Geometry: final body of the model. Coordinates: model frame, mm. A direction names the side the tool comes from. Coordinates: 2 decimals unless noted, no trailing zeros. Write each loop counter-clockwise with the first axis right and the second up, starting at its lowest first coordinate (ties: lowest second). Pieces come first, ordered by that corner, then holes.
from build123d import *

# Parameters (mm, degrees)
SKETCH1_W               = 1100
SKETCH1_H               = 500
SKETCH1_W_2             = 1000
SKETCH1_H_2             = 400
BOSS_EXTRUDE1_DEPTH     = 75
SKETCH2_W               = 50
SKETCH2_H               = 50
BOSS_EXTRUDE2_DEPTH     = 800
CUT_EXTRUDE1_DEPTH      = 1383.931668594
CUT_EXTRUDE1_DEPTH_BACK = 1383.931668594
SKETCH3_R               = 7.5


with BuildPart() as part:
    # Sketch1 → Boss-Extrude1 (new body)
    with BuildSketch(Plane(origin=(0, 0, 0), x_dir=(1, 0, 0), z_dir=(0, 1, 0))):
        Rectangle(SKETCH1_W, SKETCH1_H)
        Rectangle(SKETCH1_W_2, SKETCH1_H_2, mode=Mode.SUBTRACT)
    extrude(amount=BOSS_EXTRUDE1_DEPTH)

    # Sketch2 → Boss-Extrude2 (add)
    with BuildSketch(Plane.XZ):
        with Locations((-525, 225)):
            Rectangle(SKETCH2_W, SKETCH2_H)
        with Locations((525, 225)):
            Rectangle(SKETCH2_W, SKETCH2_H)
        with Locations((525, -225)):
            Rectangle(SKETCH2_W, SKETCH2_H)
        with Locations((-525, -225)):
            Rectangle(SKETCH2_W, SKETCH2_H)
    extrude(amount=BOSS_EXTRUDE2_DEPTH)

    # Sketch3 → Cut-Extrude1 (cut, two sides: drawn at the far end of the back side and taken through both)
    with BuildSketch(Plane.ZY.offset(550).offset(-CUT_EXTRUDE1_DEPTH_BACK)):
        with Locations(Location((0, 52.5, 0), (0, 0, 180))):
            Circle(SKETCH3_R)
    extrude(amount=CUT_EXTRUDE1_DEPTH + CUT_EXTRUDE1_DEPTH_BACK, mode=Mode.SUBTRACT)


solid = part.part
Item 1: Pin query (flat end, axial travel): pin 1 (15 mm diameter, centred on x = 525.5, z = -93, fed in from -Y). Return the tip coordinate at first contact, or that it passes through.
Derived:
pin 1: stops at y = 0
Item 2: Section A-A, the plane y = -232.5. Output: boundary loops of the cut face in (x, z), plus the area to 3 significant figures.
Derived:
outline: (-550, -250) - (-500, -250) - (-500, -200) - (-550, -200) - close; (-550, 200) - (-500, 200) - (-500, 250) - (-550, 250) - close; (500, -250) - (550, -250) - (550, -200) - (500, -200) - close; (500, 200) - (550, 200) - (550, 250) - (500, 250) - close
area: 10,000 mm2
Item 3: Section C-C, the plane x = -438. Output: boundary loops of the cut face in (y, z), plus the area to 3 significant figures.
Derived:
outline: (0, -250) - (75, -250) - (75, -200) - (0, -200) - close; (0, 200) - (75, 200) - (75, 250) - (0, 250) - close
area: 7,500 mm2
Item 4: Material intervals for probe 1 along Z at (x, y) = (516, 52); probe 2 along Y at (x, z) = (-532, 0); probe 3 along Z at (x, y) = (312, 21), sorted ascending.
Derived:
probe 1: z = -250 to -7.48, 7.48 to 250
probe 2: y = 0 to 45, 60 to 75
probe 3: z = -250 to -200, 200 to 250
Item 5: Pull-direction query (X, two-part tool) for faces 1 (the flat face through (-500, -394, -225)), 2 (the flat face through (550, -300, 205)), 3 (the flat face through (-550, -263, -205)), 4 (the flat face through (525, -394, -200)); classes: released by +X, released by -X, zero draft, split by the parting line, or undercut.
Derived:
face 1: undercut
face 2: released by +X
face 3: released by -X
face 4: zero draft
Item 6: Set-up query: faces 5 (the flat face through (-7, 37, -200)), 6 (the flat face through (-7, 0, 225)), 7 (the flat face through (-525, 0, -3)), 8 (the flat face through (-525, -800, 225)). Return all of +Z, -Z, +X, -X, +Y, -Y with unobstructed straight access to the full face (end or side cutting, diameter ignored); none if empty.
Derived:
face 5: +Y, -Y
face 6: +Z, -Z, -Y
face 7: +X, -X, -Y
face 8: +Z, -Z, +X, -X, -Y
Item 7: Section B-B, the plane z = -176. Output: boundary loops of the cut face in (x, y), plus the area to 3 significant figures.
Derived:
outline: (-550, 0) - (-500, 0) - (-500, 75) - (-550, 75) - close; (500, 0) - (550, 0) - (550, 75) - (500, 75) - close
area: 7,500 mm2
